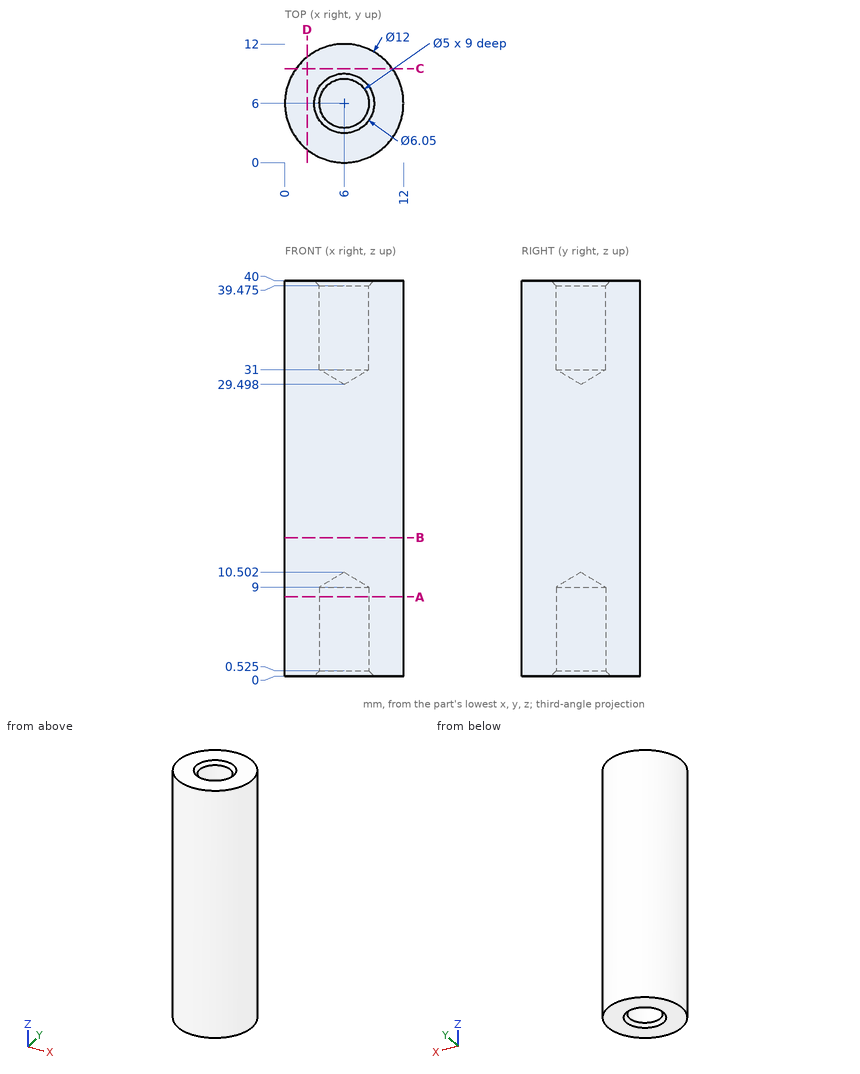
Verification items for this drawing (mm, ordinates from the low corner). Coordinates: 2 decimals unless noted, no trailing zeros. Order: outer loops, then holes, each group sorted by start corner. A loop starts at its lowest first (then second) coordinate and runs counter-clockwise, first axis right, second up. Notation, with made-up numbers: M 87.5,73 L 139.5,73 A15 cw 139.5,83 Z; hole C -9,-30 d6. An arc over 180 degrees is marked long. One line per item, written item: value. Start each with the question number.
Item 1: Depth check by flat-ended pin: P1, Ø5, axis at y = 9, z = 7, coming from the +X side; P2, Ø6, axis at x = 6, y = 6, coming from the -Z side (1 decimal). Enter the tip coordinate at first touch or a pass-through.
Item 2: Sectioned sample at B-B on z = 14. Record the cut outline in (x, y).
Item 3: Sectioned sample at D-D on x = 2.25. Record the cut outline in (y, z).
Item 4: Sectioned sample at C-C on y = 9.5. Record the cut outline in (x, z).
Item 5: Thickness scan on probe 1 along Y at (x, z) = (6, 2.75); probe 2 along Y at (x, z) = (4, 38); probe 3 along X at (y, z) = (8, 19.5). Record the ranges inside material, lowest first.
Item 6: Sectioned sample at A-A on z = 8. Record the cut outline in (x, y).
Calculated:
1. P1: x = 11.98
1. P2: z = 0
2. outline: C 6,6 d12
3. outline: M 1.32,0 L 10.68,0 L 10.68,40 L 1.32,40 Z
4. outline: M 1.13,0 L 10.87,0 L 10.87,40 L 1.13,40 Z
5. probe 1: 0 to 3.5, 8.5 to 12
5. probe 2: 0.34 to 4.5, 7.5 to 11.66
5. probe 3: 0.34 to 11.66
6. outline: C 6,6 d12; hole C 6,6 d5
